The listing builds one solid part. Answer for the finished solid, in the listing's coordinates (mm). Face numbers are marked on the shaded views. A direction names the side the tool comes from. Round coordinates to 2 decimals unless told otherwise and drop trailing zeros. Loops run counter-clockwise (first coordinate to the right, second up) from the corner with the lowest first, then second, coordinate; pieces in that order, holes last. Notation, with made-up numbers: (-34.5, -34.5) -> (-0.5, -34.5) arc R19 cw to (-0.5, -28.5) -> close; hole circle Ø8 at (57, -15). An arc over 180 degrees is marked (long way). Write each question's results on one line, items separated by ' | '. Start each with the question number.
(1) The part is cut by section A-A (z = 39.5). Determine the outline of the cut face in (x, y).
(2) The part is cut by section C-C (z = 19). Determine the outline of the cut face in (x, y).
(3) Flat-ended cylindrical pins translate along their axes: pin 1 (2 mm diameter, centred on x = -7, z = 29.79, fed in from +Y); pin 2 (10 mm diameter, centred on x = -6, z = 38, fed in from -Y); pin 3 (12 mm diameter, centred on x = -2.5, y = 1.5, fed in from -Z); pin 4 (12 mm diameter, centred on x = 1.5, y = -4.5, fed in from +Z). Find the tip coordinate at first contact, or state that the pin passes through.
(4) The part is cut by section D-D (z = 25.5). Determine the outline of the cut face in (x, y), plus the area to 3 significant figures.
(5) Determine the mould class of the marked faces 1, 2, 3 and 4 for opening direction Z: released by +Z, released by -Z, zero draft, split by the parting line, or undercut.
(6) For the marked faces 5, 6 and 7, determine the directions among +Z, -Z, +X, -X, +Y, -Y from which every point of the face is accessible in a straight line to the end or side of a thin tool.
(7) The part is cut by section B-B (y = 8). Determine the outline of the cut face in (x, z), plus the area to 3 significant figures.
(8) Straight lines are drawn through the part: probe 1 along Z at (x, y) = (-2, -20); probe 2 along X at (y, z) = (19.25, 22); probe 3 along Z at (x, y) = (14, -17). For each, find the intervals that lie inside material, in ascending order.
```python
from build123d import *

# Parameters (mm, degrees)
SKETCH1_W             = 40
SKETCH1_H             = 50
BOSS_EXTRUDE1_DEPTH   = 44
SKETCH2_R             = 5
CUT_EXTRUDE1_DEPTH    = 20
CIRPATTERN1_COUNT     = 3
M4_TAPPED_HOLE1_D     = 3.3
M4_TAPPED_HOLE1_DEPTH = 10.1
M4_TAPPED_HOLE1_TIP   = 0.991420021
SKETCH7_W             = 25
SKETCH7_H             = 8
CUT_EXTRUDE2_DEPTH    = 70.541354603
CHAMFER1_SIZE         = 2
FILLET1_R             = 5
M3_TAPPED_HOLE2_D     = 2.5
M3_TAPPED_HOLE2_DEPTH = 8.5
M3_TAPPED_HOLE2_TIP   = 0.751075774


with BuildPart() as part:
    # Sketch1 → Boss-Extrude1 (new body)
    with BuildSketch(Plane.XY):
        Rectangle(SKETCH1_W, SKETCH1_H)
    extrude(amount=BOSS_EXTRUDE1_DEPTH)

    # Sketch2 → Cut-Extrude1 (cut)
    with BuildSketch(Plane(origin=(0, 25, 0), x_dir=(1, 0, 0), z_dir=(0, 1, 0))):
        with Locations(Location((-2.5, -22, 0), (0, 0, 270))):
            Circle(SKETCH2_R)
    extrude(amount=-CUT_EXTRUDE1_DEPTH, mode=Mode.SUBTRACT)

    # Sketch3 → M3 Tapped Hole1 (revolve, cut)
    with BuildSketch(Plane(origin=(6.5, 25, 22), x_dir=(0, 0, 1), z_dir=(1, 0, 0))):
        Polygon((0, 0), (0, 8.251075774), (1.25, 7.5), (1.25, 0), align=None)
    m3_tapped_hole1 = revolve(axis=Axis((6.5, 31.35, 22), (0, -1, 0)), mode=Mode.SUBTRACT)

    # CirPattern1: M3 Tapped Hole1 ×3 about axis
    cirpattern1_axis = Axis((-2.5, 0, 22), (0, 1, 0))
    for i in range(1, CIRPATTERN1_COUNT):
        add(m3_tapped_hole1.rotate(cirpattern1_axis, i * 360 / CIRPATTERN1_COUNT), mode=Mode.SUBTRACT)

    # M4 Tapped Hole1
    with Locations(Plane(origin=(0, -25, 0), x_dir=(-1, 0, 0), z_dir=(0, -1, 0))):
        with Locations((-14, -32), (2, -32), (-14, -12), (2, -12)):
            Hole(M4_TAPPED_HOLE1_D / 2, depth=M4_TAPPED_HOLE1_DEPTH)
            with Locations((0, 0, -(M4_TAPPED_HOLE1_DEPTH + M4_TAPPED_HOLE1_TIP / 2))):  # 118° drill point
                Cone(0, M4_TAPPED_HOLE1_D / 2, M4_TAPPED_HOLE1_TIP, mode=Mode.SUBTRACT)

    # Sketch7 → Cut-Extrude2 (cut, through all)
    with BuildSketch(Plane.XZ.offset(25)):
        with Locations((0, 40)):
            Rectangle(SKETCH7_W, SKETCH7_H)
        with Locations((0, 4)):
            Rectangle(SKETCH7_W, SKETCH7_H)
    extrude(amount=-CUT_EXTRUDE2_DEPTH, mode=Mode.SUBTRACT)

    # Chamfer1
    chamfer1_edges = [part.edges().sort_by_distance(p)[0] for p in [
        (-16.25, -25, 44),
        (-16.25, -25, 0),
        (-16.25, 25, 44),
        (16.25, -25, 44),
        (16.25, 25, 0),
        (16.25, -25, 0),
        (-16.25, 25, 0),
        (16.25, 25, 44),
    ]]
    chamfer(chamfer1_edges, length=CHAMFER1_SIZE)

    # Fillet1
    fillet1_edges = [part.edges().sort_by_distance(p)[0] for p in [
        (12.5, 0, 36),
        (-12.5, 0, 36),
        (12.5, 0, 8),
        (-12.5, 0, 8),
    ]]
    fillet(fillet1_edges, radius=FILLET1_R)

    # M3 Tapped Hole2
    with Locations(Plane(origin=(0, 25, 0), x_dir=(1, 0, 0), z_dir=(0, 1, 0))):
        with Locations((16.25, -31), (16.25, -13)):
            Hole(M3_TAPPED_HOLE2_D / 2, depth=M3_TAPPED_HOLE2_DEPTH)
            with Locations((0, 0, -(M3_TAPPED_HOLE2_DEPTH + M3_TAPPED_HOLE2_TIP / 2))):  # 118° drill point
                Cone(0, M3_TAPPED_HOLE2_D / 2, M3_TAPPED_HOLE2_TIP, mode=Mode.SUBTRACT)


solid = part.part
```
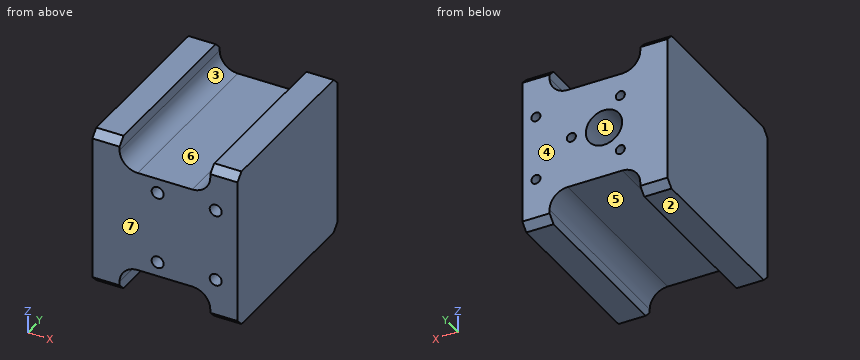
Checked values:
1) outline: (-20, -25) -> (-12.27, -25) -> (-12.27, 25) -> (-20, 25) -> close; (12.27, -25) -> (20, -25) -> (20, 25) -> (12.27, 25) -> close
2) outline: (-20, -25) -> (20, -25) -> (20, 25) -> (1.5, 25) -> (1.5, 5) -> (-6.5, 5) -> (-6.5, 25) -> (-20, 25) -> close
3) pin 1: stops at y = 17.35 | pin 2: stops at y = -25 | pin 3: stops at z = 7.9 | pin 4: stops at z = 36
4) outline: (-20, -25) -> (20, -25) -> (20, 25) -> (1.07, 25) -> (1.07, 5) -> (-6.07, 5) -> (-6.07, 25) -> (-20, 25) -> close | area: 1,860 mm2
5) face 1: undercut | face 2: released by -Z | face 3: released by +Z | face 4: zero draft
6) face 5: -Z, +Y, -Y | face 6: +Z, +Y, -Y | face 7: +Z, -Z, +X, -X, -Y
7) outline: (-20, 0) -> (-12.5, 0) -> (-12.5, 3) arc R5 cw to (-7.5, 8) -> (7.5, 8) arc R5 cw to (12.5, 3) -> (12.5, 0) -> (20, 0) -> (20, 44) -> (12.5, 44) -> (12.5, 41) arc R5 cw to (7.5, 36) -> (-7.5, 36) arc R5 cw to (-12.5, 41) -> (-12.5, 44) -> (-20, 44) -> close; hole circle Ø10 at (-2.5, 22) | area: 1,300 mm2
8) probe 1: z = 8 to 10.35, 13.65 to 30.35, 33.65 to 36 | probe 2: x = -20 to -7.5, 2.5 to 5.25, 7.75 to 20 | probe 3: z = 0 to 10.35, 13.65 to 30.35, 33.65 to 44
